Design review of the part built by this model. Coordinates are the model's own, in mm. A direction names the side the tool comes from. Give positions to 0.01 mm unless a question says otherwise; leave off trailing zeros. Loops run counter-clockwise (first coordinate to the right, second up) from the corner with the lowest first, then second, coordinate; pieces in that order, holes last. Notation, with made-up numbers: (2.5, 13.5) - (56.5, 13.5) arc R30 ccw to (56.5, 40.5) - close; hole circle Ø7 at (-33.5, 54.5). An arc over 180 degrees is marked (long way). Write each question's results on one line, items separated by ' | '.
from build123d import *

# Parameters (mm, degrees)
BOSS_EXTRUDE1_DEPTH    = 1116
SKETCH2_W              = 92.475127077
SKETCH2_H              = 38.646657261
SKETCH2_W_2            = 90.397253408
SKETCH2_H_2            = 44.857464027
CUT_EXTRUDE1_DEPTH     = 1116
SKETCH3_R              = 4
CUT_EXTRUDE2_DEPTH     = 1116
FILLET1_R              = 5
M10_TAPPED_HOLE1_D     = 8.5
M10_TAPPED_HOLE1_DEPTH = 24.5
M10_TAPPED_HOLE1_TIP   = 2.553657631


with BuildPart() as part:
    # Sketch1 → Boss-Extrude1 (new body)
    with BuildSketch(Plane.XY):
        with BuildLine():
            Line((0, 0), (37, 0))
            ThreePointArc((37, 0), (42.656854249, -2.343145751), (45, -8))
            Line((45, -8), (45, -52))
            ThreePointArc((45, -52), (42.656854249, -57.656854249), (37, -60))
            Line((37, -60), (0, -60))
            Line((0, -60), (0, -55))
            Line((0, -55), (37, -55))
            ThreePointArc((37, -55), (39.121320344, -54.121320344), (40, -52))
            Line((40, -52), (40, -8))
            ThreePointArc((40, -8), (39.121320344, -5.878679656), (37, -5))
            Line((37, -5), (0, -5))
            Line((0, -5), (0, 0))
        make_face()
    extrude(amount=BOSS_EXTRUDE1_DEPTH)

    # Sketch2 → Cut-Extrude1 (cut)
    with BuildSketch(Plane.ZY):
        with Locations((1105.237563539, -71.323328631)):
            Rectangle(SKETCH2_W, SKETCH2_H)
        with Locations((11.801373296, -74.428732013)):
            Rectangle(SKETCH2_W_2, SKETCH2_H_2)
    extrude(amount=-CUT_EXTRUDE1_DEPTH, mode=Mode.SUBTRACT)

    # Sketch3 → Cut-Extrude2 (cut)
    with BuildSketch(Plane(origin=(0, -55, 0), x_dir=(1, 0, 0), z_dir=(0, 1, 0))):
        with Locations(Location((12.5, -1024, 0), (0, 0, 270))):
            Circle(SKETCH3_R)
    extrude(amount=-CUT_EXTRUDE2_DEPTH, mode=Mode.SUBTRACT)

    # Fillet1
    fillet1_edges = [part.edges().sort_by_distance(p)[0] for p in [
        (42.5, -52, 0),
        (42.5, -52, 1116),
    ]]
    fillet(fillet1_edges, radius=FILLET1_R)

    # M10 Tapped Hole1
    with Locations(Plane(origin=(0, -55, 0), x_dir=(1, 0, 0), z_dir=(0, 1, 0))):
        with Locations((12.5, -1024)):
            Hole(M10_TAPPED_HOLE1_D / 2, depth=M10_TAPPED_HOLE1_DEPTH)
            with Locations((0, 0, -(M10_TAPPED_HOLE1_DEPTH + M10_TAPPED_HOLE1_TIP / 2))):  # 118° drill point
                Cone(0, M10_TAPPED_HOLE1_D / 2, M10_TAPPED_HOLE1_TIP, mode=Mode.SUBTRACT)


solid = part.part
(1) Insertion check: P1, Ø5, axis at y = -17.5, z = 167, coming from the -X side; P2, Ø2.5, axis at x = 15, y = -55, coming from the -Z side; P3, Ø1.5, axis at x = 41.5, z = 29, coming from the -Y side. Each pin has a flat end and moves straight along its axis. Give the tip position at first contact, or say it passes through.
Answers below:
P1: x = 40 | P2: z = 57 | P3: y = -52
(2) Take a section at B-B on z = 556. Give the boundary of the cut face in (x, y).
Answers below:
outline: (0, -60) - (37, -60) arc R8 ccw to (45, -52) - (45, -8) arc R8 ccw to (37, 0) - (0, 0) - (0, -5) - (37, -5) arc R3 cw to (40, -8) - (40, -52) arc R3 cw to (37, -55) - (0, -55) - close
(3) Take a section at A-A on x = 26. Give the boundary of the cut face in (y, z), plus the area to 3 significant figures.
Answers below:
outline: (-60, 57) - (-55, 57) - (-55, 1059) - (-60, 1059) - close; (-5, 0) - (0, 0) - (0, 1116) - (-5, 1116) - close | area: 10,600 mm2
(4) Tool access review of faces 4 (the flat face through (40, -30, 550)), 5 (the flat face through (41, -15, 0)): name each direction out of +Z, -Z, +X, -X, +Y, -Y from which nothing blocks a thin tool from reaching the whole face with its end or side.
Answers below:
face 4: +Z, -Z, -X | face 5: -Z, +X, -X, +Y, -Y
(5) Draft analysis for pull direction Y (two halves, no side actions). For faces 1 (the flat face through (18, 0, 550)), 2 (the flat face through (18, -55, 551)), 3 (the flat face through (45, -30, 550)), state which applies: pulls with the +Y half, pulls with the -Y half, needs draft (parallel to the pull), parting line crosses it, or undercut.
Answers below:
face 1: pulls with the +Y half | face 2: undercut | face 3: needs draft
(6) Wall thickness on line 1 along Y through (x, z) = (13.5, 416); line 2 along Z through (x, y) = (12.5, -57.4); line 3 along X through (y, z) = (-39, 315.5): over which ranges is each line inside the solid? List them lowest first. Write a range as from..to.
Answers below:
line 1: -60..-55, -5..0 | line 2: 57..1019.75, 1028.25..1059 | line 3: 40..45
